```python
from build123d import *

# Parameters (mm, degrees)
MEMBER_1_DEPTH          = 60
SKETCH_3_W              = 60
SKETCH_3_H              = 15
CUT_EXTRUDE_1_DEPTH     = 177.068168617
SKETCH_4_W              = 60
SKETCH_4_H              = 4
CUT_EXTRUDE_2_DEPTH     = 171.660481659
HOLE_WIZARD_6_5_6_5_1_D = 6.5
FILLET_1_R              = 3
HOLE_WIZARD_8_5_8_5_1_D = 8.5


with BuildPart() as part:
    # Sketch1 → Member 1 (new body)
    with BuildSketch(Plane(origin=(0, 0, 0), x_dir=(0, 0, -1), z_dir=(1, 0, 0))):
        with BuildLine():
            Line((0, 0), (0, 150))
            ThreePointArc((0, 150), (5.656854249, 147.656854249), (8, 142))
            Line((8, 142), (8, 13))
            ThreePointArc((8, 13), (9.464466094, 9.464466094), (13, 8))
            Line((13, 8), (62, 8))
            ThreePointArc((62, 8), (67.656854249, 5.656854249), (70, 0))
            Line((70, 0), (0, 0))
        make_face()
    extrude(amount=MEMBER_1_DEPTH)

    # 草图3 → 切除-拉伸1 (cut, through all)
    with BuildSketch(Plane.XZ):
        with Locations((30, -62.5)):
            Rectangle(SKETCH_3_W, SKETCH_3_H)
    extrude(amount=-CUT_EXTRUDE_1_DEPTH, mode=Mode.SUBTRACT)

    # 草图4 → 切除-拉伸2 (cut, through all)
    with BuildSketch(Plane.XY):
        with Locations((30, 148)):
            Rectangle(SKETCH_4_W, SKETCH_4_H)
    extrude(amount=-CUT_EXTRUDE_2_DEPTH, mode=Mode.SUBTRACT)

    # Ø6.5 (6.5) 直径孔1 (through all)
    with Locations(Plane(origin=(0, 0, -8), x_dir=(-1, 0, 0), z_dir=(0, 0, -1))):
        with Locations((-45, 135.5), (-15, 135.5), (-45, 80.5), (-15, 80.5)):
            Hole(HOLE_WIZARD_6_5_6_5_1_D / 2)

    # 圆角1
    fillet_1_edges = [part.edges().sort_by_distance(p)[0] for p in [
        (0, 4, -55),
        (60, 4, -55),
    ]]
    fillet(fillet_1_edges, radius=FILLET_1_R)

    # Ø8.5 (8.5) 直径孔1 (through all)
    with Locations(Plane(origin=(0, 8, 0), x_dir=(1, 0, 0), z_dir=(0, 1, 0))):
        with Locations((15, 30), (45, 30)):
            Hole(HOLE_WIZARD_8_5_8_5_1_D / 2)


solid = part.part
```
Can you work these out from the model? Positions are in its coordinate system, mm. A direction names the side the tool comes from. Give positions to 0.01 mm unless a question says otherwise; leave off trailing zeros. Loops run counter-clockwise (first coordinate to the right, second up) from the corner with the lowest first, then second, coordinate; pieces in that order, holes last. Notation, with made-up numbers: M -22,26.25 L 31,26.25 A23 ccw 31,63.25 Z; hole C 49.5,8 d2. An arc over 180 degrees is marked long. One line per item, written item: value.
(1) Suppose I cut it at C-C on x = 53.5. List the corners of the cut face in (y, z) for me, plus the area to 3 significant figures.
Returned:
outline: M 0,-55 L 8,-55 L 8,-13 A5 cw 13,-8 L 142,-8 A8 ccw 146,-6.93 L 146,0 L 0,0 Z
area: 1,550 mm^2
(2) Suppose I cut it at A-A on x = 45. List the corners of the cut face in (y, z) for me.
Returned:
outline: M 0,-55 L 8,-55 L 8,-34.25 L 0,-34.25 Z; M 0,-25.75 L 8,-25.75 L 8,-13 A5 cw 13,-8 L 77.25,-8 L 77.25,0 L 0,0 Z; M 83.75,-8 L 132.25,-8 L 132.25,0 L 83.75,0 Z; M 138.75,-8 L 142,-8 A8 ccw 146,-6.93 L 146,0 L 138.75,0 Z
(3) I need wall thicknesses on line 1 (Y direction, x = 45, z = -2); line 2 (X direction, y = 5.25, z = -30); line 3 (X direction, y = 135.5, z = -6.5). Which ranges of each line are inside material? Lowest first, please.
Returned:
line 1: 0 to 77.25, 83.75 to 132.25, 138.75 to 146
line 2: 0 to 10.75, 19.25 to 40.75, 49.25 to 60
line 3: 0 to 11.75, 18.25 to 41.75, 48.25 to 60
(4) Suppose I cut it at D-D on z = -15.5. List the corners of the cut face in (x, y) for me, plus the area to 3 significant figures.
Returned:
outline: M 0,0 L 60,0 L 60,8 L 0,8 Z
area: 480 mm^2
(5) We'd pull the mould along Z, two halves only. Please class faces 1 (the face through (49.246, 3.944, -30.187)), 2 (the face through (30, 0, -28)), 3 (the face through (30, 4, -55)): released by +Z, released by -Z, zero draft, split by the parting line, or undercut.
Returned:
face 1: undercut
face 2: zero draft
face 3: released by -Z
(6) Will these pins go through, and if not, where does the flat tip stop? pin 1 (1.5 mm diameter, centred on x = 41, z = -29.5, fed in from +Y); pin 2 (8 mm diameter, centred on x = 16.5, y = 111.5, fed in from +Z); pin 3 (18 mm diameter, centred on x = 39.5, y = 104, fed in from -Z).
Returned:
pin 1: y = 8
pin 2: z = 0
pin 3: z = -8
(7) Which directions (+Z, -Z, +X, -X, +Y, -Y) give clear straight access to the entire face, cutting with the end or side of a thin tool? Please do faces 4 (the face through (30, 146, -3)), 5 (the face through (30, 8, -34)).
Returned:
face 4: +Z, -Z, +X, -X, +Y
face 5: -Z, +X, -X, +Y
(8) Suppose I cut it at B-B on y = 135.5. List the corners of the cut face in (x, z) for me.
Returned:
outline: M 0,-8 L 11.75,-8 L 11.75,0 L 0,0 Z; M 18.25,-8 L 41.75,-8 L 41.75,0 L 18.25,0 Z; M 48.25,-8 L 60,-8 L 60,0 L 48.25,0 Z
